from build123d import *

# Parameters (mm, degrees)
SKETCH1_R           = 5
BOSS_EXTRUDE1_DEPTH = 87
SKETCH2_R           = 3
CUT_EXTRUDE1_DEPTH  = 10


with BuildPart() as part:
    # Sketch1 → Boss-Extrude1 (new, symmetric)
    with BuildSketch(Plane.XY):
        Circle(SKETCH1_R)
    extrude(amount=BOSS_EXTRUDE1_DEPTH, both=True)

    # Sketch2 → Cut-Extrude1 (cut)
    with BuildSketch(Plane.XY.offset(87)):
        Circle(SKETCH2_R)
    cut_extrude1 = extrude(amount=-CUT_EXTRUDE1_DEPTH, mode=Mode.SUBTRACT)

    # Mirror1: Cut-Extrude1 across plane
    add(cut_extrude1.mirror(Plane.XY), mode=Mode.SUBTRACT)


solid = part.part
Build history of the part. All positions in model axes, mm. A direction names the side the tool comes from. Round coordinates to 2 decimals unless told otherwise and drop trailing zeros. Write each loop counter-clockwise with the first axis right and the second up, starting at its lowest first coordinate (ties: lowest second). Pieces come first, ordered by that corner, then holes. Notation, with made-up numbers: M -10,-36.75 L 8,-36.75 A27 ccw 8,-3.75 Z; hole C -35.5,54 d9. An arc over 180 degrees is marked long. Answer in a Markdown table with one row per item.
1. Saw through at C-C (z = 1). List the corners of the cut face in (x, y).
Geometry check:
| item | result |
|---|---|
| outline | C 0,0 d10 |
2. Flat gauge pins, fed straight in: P1, Ø3, axis at x = -2.5, z = -10, coming from the +Y side; P2, Ø3.5, axis at x = 0, y = 0, coming from the -Z side; P3, Ø5, axis at x = 0, y = 0, coming from the +Z side. Where does each tip first touch, or does it go through?
Geometry check:
| item | result |
|---|---|
| P1 | y = 4.9 |
| P2 | z = -77 |
| P3 | z = 77 |
3. Mould opens along Y. For faces 4 (the face through (0, 0, -77)), 5 (the face through (-1.08, -4.88, 1.22)), 6 (the face through (-0.1, -3.3, 87)) say: +Y half, -Y half, draft (parallel to the pull), parting line (faces both ways), or undercut.
Geometry check:
| item | result |
|---|---|
| face 4 | undercut |
| face 5 | parting line |
| face 6 | draft |
4. Probe L1, parallel to Y at x = 0, z = 82.5; L2, parallel to Z at x = -1.5, y = 0; L3, parallel to Y at x = 4, z = -48.5. List the from-to ranges inside material, lowest first. Write a range as [from, to].
Geometry check:
| item | result |
|---|---|
| L1 | [-5, -3], [3, 5] |
| L2 | [-77, 77] |
| L3 | [-3, 3] |
5. Which spindle directions (+Z, -Z, +X, -X, +Y, -Y) get a long thin tool onto all of the face, cutting with end or side? Do faces 1 (the face through (-3, 0, -82)), 2 (the face through (-0.1, -3.3, -87)), 3 (the face through (0, 0, 77)). Say none if no direction does.
Geometry check:
| item | result |
|---|---|
| face 1 | -Z |
| face 2 | -Z, +X, -X, +Y, -Y |
| face 3 | +Z |
6. Saw through at A-A (y = 0). List the corners of the cut face in (x, z), and give its area (3 significant figures).
Geometry check:
| item | result |
|---|---|
| outline | M -5,-87 L -3,-87 L -3,-77 L 3,-77 L 3,-87 L 5,-87 L 5,87 L 3,87 L 3,77 L -3,77 L -3,87 L -5,87 Z |
| area | 1,620 mm2 |
